```python
from build123d import *

# Parameters (mm, degrees)
SKETCH2_W          = 6.5
SKETCH2_H          = 1.083333334
CUT_EXTRUDE1_DEPTH = 2


with BuildPart() as part:
    # Sketch1 → Revolve1 (revolve)
    with BuildSketch(Plane.XY, mode=Mode.PRIVATE) as revolve1_sk:
        with BuildLine():
            Line((-10, 0), (-10, 4.85))
            Line((-10, 4.85), (-9.5, 5.35))
            Line((-9.5, 5.35), (-9.5, 5.959415537))
            ThreePointArc((-9.5, 5.959415537), (-9.3567275, 6.309766063), (-9.009018036, 6.459334205))
            ThreePointArc((-9.009018036, 6.459334205), (-5.001066402, 6.499497864), (-0.992985972, 6.475400495))
            ThreePointArc((-0.992985972, 6.475400495), (-0.643975412, 6.326514493), (-0.5, 5.975449694))
            Line((-0.5, 5.975449694), (-0.5, 5.35))
            Line((-0.5, 5.35), (0, 4.85))
            Line((0, 4.85), (0, 2.5))
            Line((0, 2.5), (12.5095, 2.5))
            Line((12.5095, 2.5), (13, 2.0095))
            Line((13, 2.0095), (13, 0))
            Line((13, 0), (-10, 0))
        make_face()
    revolve(revolve1_sk.sketch.rotate(Axis((13, 0, 0), (-1, 0, 0)), 270), axis=Axis((13, 0, 0), (-1, 0, 0)))

    # Sketch2 → Cut-Extrude1 (cut)
    with BuildSketch(Plane.ZY.offset(10)):
        Rectangle(SKETCH2_W, SKETCH2_H)
    extrude(amount=-CUT_EXTRUDE1_DEPTH, mode=Mode.SUBTRACT)


solid = part.part
```
Check sheet for the modelled part. Datum: model origin and axes. Units: mm. A direction names the side the tool comes from. Give positions to 0.01 mm unless a question says otherwise; leave off trailing zeros. Order: outer loops, then holes, each group sorted by start corner. A loop starts at its lowest first (then second) coordinate and runs counter-clockwise, first axis right, second up. Notation, with made-up numbers: M 74.25,-6.5 L 96.25,-6.5 A25 cw 96.25,25.5 Z; hole C 87.5,78 d5. An arc over 180 degrees is marked long. Answer in a Markdown table with one row per item. Add a question column.
Q1. Sectioned sample at A-A, the plane x = 2.5. Record the boundary of the cut face in (y, z).
Q2. Thickness scan on L1, parallel to X at y = -5, z = 3; L2, parallel to X at y = -3.5, z = 0.75; L3, parallel to Y at x = -6.5, z = 0.75. Record the ranges inside material, lowest first.
Q3. Release check for a two-part mould opening along Z. For faces 1 (the flat face through (-9.5, 4, 4)), 2 (the flat face through (-9, 0.542, 0)), 3 (the flat face through (-9, 0, 3.25)), 4 (the cylindrical face through (6.34, -2.44, -0.54)) record: released by +Z, released by -Z, zero draft, split by the parting line, or undercut.
Q4. Gauge pin test, flat ends, axial feed: pin 1 Ø0.9 at (x, y) = (-9.5, 0) entering from -Z; pin 2 Ø1 at (x, y) = (-7.5, 3.5) entering from -Z; pin 3 Ø2 at (x, z) = (-1, 3.5) entering from -Y. Record the tip position at first contact, or that the pin passes through.
Q5. Access from +Z, -Z, +X, -X, +Y, -Y to the whole of each face (thin tool, end or side, straight path). Record for faces 5 (the flat face through (-9, -0.542, 0)), 6 (the flat face through (0, -2, 2)), 7 (the flat face through (-10, -1, 0)).
Verdict:
| question | item | result |
|---|---|---|
| 1 | outline | C 0,0 d5 |
| 2 | L1 | -9.5 to -0.5 |
| 2 | L2 | -10 to 0 |
| 2 | L3 | -6.45 to 6.45 |
| 3 | face 1 | zero draft |
| 3 | face 2 | undercut |
| 3 | face 3 | undercut |
| 3 | face 4 | split by the parting line |
| 4 | pin 1 | z = -6.46 |
| 4 | pin 2 | z = -5.75 |
| 4 | pin 3 | y = -5.97 |
| 5 | face 5 | -X |
| 5 | face 6 | +X |
| 5 | face 7 | +Z, -Z, -X, +Y, -Y |
